The model under review builds one solid part; all positions refer to its coordinate system, in mm. Face numbers are marked on the shaded views. A direction names the side the tool comes from. Coordinates: 2 decimals unless noted, no trailing zeros. Order: outer loops, then holes, each group sorted by start corner. A loop starts at its lowest first (then second) coordinate and runs counter-clockwise, first axis right, second up. Notation, with made-up numbers: (75, 25) -> (105, 25) arc R21 cw to (105, 48) -> close; hole circle Ø1 at (10, 88). An arc over 180 degrees is marked (long way). Use one line per item in the form item = value.
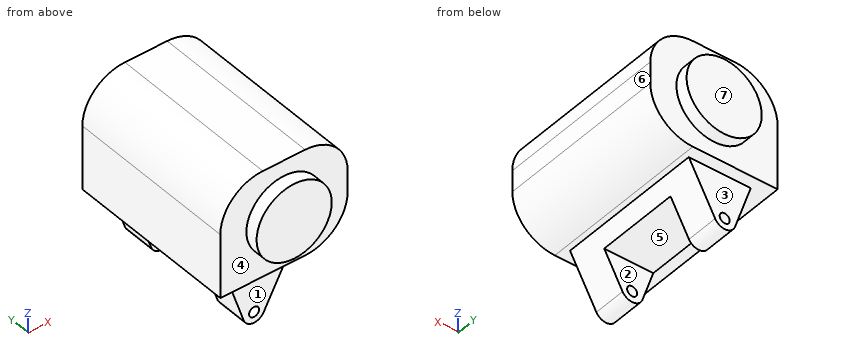
from build123d import *

# Parameters (mm, degrees)
SKETCH1_W           = 29.956211672
SKETCH1_H           = 40.65774509
BOSS_EXTRUDE1_DEPTH = 25
SKETCH2_R           = 1.179493096
BOSS_EXTRUDE2_DEPTH = 17.5
FILLET1_R           = 10
SKETCH3_R           = 8.841541065
BOSS_EXTRUDE3_DEPTH = 3
BOSS_EXTRUDE4_START = 3
SKETCH4_R           = 8.841541065
BOSS_EXTRUDE4_DEPTH = 3
SKETCH5_W           = 18.672217178
SKETCH5_H           = 19.553012946
CUT_EXTRUDE1_DEPTH  = 28


with BuildPart() as part:
    # Sketch1 → Boss-Extrude1 (new body)
    with BuildSketch(Plane.XY):
        with Locations((-25.008704873, 0)):
            Rectangle(SKETCH1_W, SKETCH1_H)
    extrude(amount=BOSS_EXTRUDE1_DEPTH)

    # Sketch2 → Boss-Extrude2 (add, symmetric)
    with BuildSketch(Plane(origin=(0, 0, -4), x_dir=(1, 0, 0), z_dir=(0, -1, 0))):
        with BuildLine():
            Line((-32.216437007, -7.03254357), (-35.914043193, 4))
            Line((-35.914043193, 4), (-21.345745646, 4))
            Line((-21.345745646, 4), (-27.542475863, -7.438106205))
            ThreePointArc((-27.542475863, -7.438106205), (-30.012436117, -8.767867117), (-32.216437007, -7.03254357))
        make_face()
        with Locations(Location((-29.791335202, -6.219759883, 0), (0, 0, 270))):
            Circle(SKETCH2_R, mode=Mode.SUBTRACT)
    extrude(amount=BOSS_EXTRUDE2_DEPTH, both=True)

    # Fillet1
    fillet1_edges = [part.edges().sort_by_distance(p)[0] for p in [
        (-39.986810709, 0, 25),
        (-10.030599037, 0, 25),
        (-10.030599037, 0, 0),
    ]]
    fillet(fillet1_edges, radius=FILLET1_R)

    # Sketch3 → Boss-Extrude3 (add)
    with BuildSketch(Plane(origin=(0, -20.328872545, 0), x_dir=(-1, 0, 0), z_dir=(0, -1, 0))):
        with Locations(Location((25.008704873, -12.5, 0), (0, 0, 90))):
            Circle(SKETCH3_R)
    extrude(amount=BOSS_EXTRUDE3_DEPTH)

    # Sketch4 → Boss-Extrude4 (add)
    with BuildSketch(Plane(origin=(0, 20.328872545, 0), x_dir=(1, 0, 0), z_dir=(0, 1, 0)).offset(BOSS_EXTRUDE4_START)):
        with Locations(Location((-25.008704873, -12.5, 0), (0, 0, 90))):
            Circle(SKETCH4_R)
    extrude(amount=-BOSS_EXTRUDE4_DEPTH)

    # Sketch5 → Cut-Extrude1 (cut)
    with BuildSketch(Plane.ZY.offset(39.986810709)):
        with Locations((-12.777441663, 0)):
            Rectangle(SKETCH5_W, SKETCH5_H)
    extrude(amount=-CUT_EXTRUDE1_DEPTH, mode=Mode.SUBTRACT)


solid = part.part
Item 1: We need section C-C (z = 12.5). Write out the cut boundary in (x, y), plus the area to 3 significant figures.
Results found:
outline = (-39.99, -20.33) -> (-33.85, -20.33) -> (-33.85, -23.33) -> (-16.17, -23.33) -> (-16.17, -20.33) -> (-10.03, -20.33) -> (-10.03, 20.33) -> (-16.17, 20.33) -> (-16.17, 23.33) -> (-33.85, 23.33) -> (-33.85, 20.33) -> (-39.99, 20.33) -> close
area = 1,320 mm²
Item 2: We need section D-D (y = -12.5). Write out the cut boundary in (x, z), plus the area to 3 significant figures.
Results found:
outline = (-39.99, 0) -> (-35.91, 0) -> (-32.22, -11.03) arc R2.56 ccw to (-27.54, -11.44) -> (-21.35, 0) -> (-20.03, 0) arc R10 ccw to (-10.03, 10) -> (-10.03, 15) arc R10 ccw to (-20.03, 25) -> (-29.99, 25) arc R10 ccw to (-39.99, 15) -> close; hole circle Ø2.36 at (-29.79, -10.22)
area = 794 mm²
Item 3: Clearance check with flat-ended pins moving along their axes: pin 1 (4.5 mm diameter, centred on x = -31, z = -6.5, fed in from -Y); pin 2 (4 mm diameter, centred on y = -16, z = 0.5, fed in from +X); pin 3 (6 mm diameter, centred on x = -30, y = 3.5, fed in from -Z). State where each tip first meets the part, or that it passes through.
Results found:
pin_1 = -17.5
pin_2 = -13.42
pin_3 = -3.44
Item 4: Draft analysis for pull direction Y (two halves, no side actions). For the marked faces 5, 6 and 7, state which applies: released by +Y, released by -Y, zero draft, split by the parting line, or undercut.
Results found:
face_5 = undercut
face_6 = zero draft
face_7 = released by +Y
Item 5: Tool access review of the marked faces 1, 2, 3 and 4: name each direction out of +Z, -Z, +X, -X, +Y, -Y from which nothing blocks a thin tool from reaching the whole face with its end or side.
Results found:
face_1 = -Z, +X, -X, -Y
face_2 = -Z, +X, -X
face_3 = -Z, +X, -X, +Y
face_4 = -Y
Item 6: We need section B-B (y = -6.5). Write out the cut boundary in (x, z), plus the area to 3 significant figures.
Results found:
outline = (-39.99, 0) -> (-35.91, 0) -> (-34.76, -3.44) -> (-23.21, -3.44) -> (-21.35, 0) -> (-20.03, 0) arc R10 ccw to (-10.03, 10) -> (-10.03, 15) arc R10 ccw to (-20.03, 25) -> (-29.99, 25) arc R10 ccw to (-39.99, 15) -> close
area = 729 mm²
Item 7: To check wall thickness, follow L1, parallel to Y at x = -24, z = 1; L2, parallel to Z at x = -30, y = 7; L3, parallel to Z at x = -29, y = 15. State the ranges of each line that lie inside material, in increasing order. Write a range as from..to.
Results found:
L1 = -20.33..20.33
L2 = -3.44..25
L3 = -12.65..-11.09, -9.35..25
Item 8: We need section A-A (z = -5.5). Write out the cut boundary in (x, y).
Results found:
outline = (-34.07, -17.5) -> (-24.33, -17.5) -> (-24.33, -9.78) -> (-34.07, -9.78) -> close; (-34.07, 9.78) -> (-24.33, 9.78) -> (-24.33, 17.5) -> (-34.07, 17.5) -> close
